from build123d import *

# Parameters (mm, degrees)
SKETCH1_R           = 20.5
BOSS_EXTRUDE1_DEPTH = 25
CHAMFER1_SIZE       = 0.5
SKETCH5_R           = 16.25
CUT_EXTRUDE1_DEPTH  = 20
CHAMFER2_SIZE       = 0.5
SKETCH6_R           = 10.5
CUT_EXTRUDE2_DEPTH  = 31


with BuildPart() as part:
    # Sketch1 → Boss-Extrude1 (new body)
    with BuildSketch(Plane.XY):
        Circle(SKETCH1_R)
    extrude(amount=BOSS_EXTRUDE1_DEPTH)

    # Chamfer1
    chamfer1_edges = [part.edges().sort_by_distance(p)[0] for p in [
        (-20.5, 0, 0),
        (-20.5, 0, 25),
    ]]
    chamfer(chamfer1_edges, length=CHAMFER1_SIZE)

    # Sketch5 → Cut-Extrude1 (cut)
    with BuildSketch(Plane.XY.offset(25)):
        Circle(SKETCH5_R)
    extrude(amount=-CUT_EXTRUDE1_DEPTH, mode=Mode.SUBTRACT)

    # Chamfer2
    chamfer2_edges = [part.edges().sort_by_distance(p)[0] for p in [
        (-16.25, 0, 25),
    ]]
    chamfer(chamfer2_edges, length=CHAMFER2_SIZE)

    # Sketch6 → Cut-Extrude2 (cut)
    with BuildSketch(Plane(origin=(0, 0, 0), x_dir=(-1, 0, 0), z_dir=(0, 0, -1))):
        Circle(SKETCH6_R)
    extrude(amount=-CUT_EXTRUDE2_DEPTH, mode=Mode.SUBTRACT)


solid = part.part
The listing builds one solid part. Answer for the finished solid, in the listing's coordinates (mm). A direction names the side the tool comes from. Coordinates: 2 decimals unless noted, no trailing zeros. Loops run counter-clockwise (first coordinate to the right, second up) from the corner with the lowest first, then second, coordinate; pieces in that order, holes last. Notation, with made-up numbers: (4.5, 17.25) -> (45.5, 17.25) arc R9 cw to (45.5, 31.25) -> close; hole circle Ø11 at (-34.75, -22). An arc over 180 degrees is marked (long way). Answer in a Markdown table with one row per item. Add a question column.
1. The part is cut by section C-C, the plane z = 2.75. Write down the section's boundary in (x, y), then the cut area to 3 significant figures.
2. The part is cut by section D-D, the plane z = 18.25. Write down the section's boundary in (x, y), then the cut area to 3 significant figures.
3. Determine the mould class of faces 1 (the cylindrical face through (-4.444, -20.013, 12.332)), 2 (the flat face through (9, -9, 0)), 3 (the cylindrical face through (15.5, 4.88, 14.89)) for opening direction X: +X half, -X half, draft (parallel to the pull), parting line (faces both ways), or undercut.
4. Consider line 1 (Y direction, x = 0, z = 1); line 2 (Y direction, x = 0, z = 11.5); line 3 (Z direction, x = -14, y = -0.5). Determine where each line is inside the solid, lowest interval first. Write a range as [from, to].
5. For faces 4 (the cylindrical face through (-10, 3.2, 2.5)), 5 (the flat face through (11, 0, 5)), determine the directions among +Z, -Z, +X, -X, +Y, -Y from which every point of the face is accessible in a straight line to the end or side of a thin tool.
6. Flat-ended cylindrical pins translate along their axes: P1, Ø16, axis at x = 2.5, y = -5, coming from the +Z side; P2, Ø5, axis at y = 6, z = 21, coming from the +X side; P3, Ø3, axis at x = 14.5, z = 21, coming from the +Y side; P4, Ø6, axis at x = 16, y = -2, coming from the +Z side. Find the tip coordinate at first contact, or state that the pin passes through.
7. The part is cut by section A-A, the plane y = 0. Write down the section's boundary in (x, z).
Answer below:
| question | item | result |
|---|---|---|
| 1 | outline | circle Ø41 at (0, 0); hole circle Ø21 at (0, 0) |
| 1 | area | 974 mm2 |
| 2 | outline | circle Ø41 at (0, 0); hole circle Ø32.5 at (0, 0) |
| 2 | area | 491 mm2 |
| 3 | face 1 | parting line |
| 3 | face 2 | draft |
| 3 | face 3 | undercut |
| 4 | line 1 | [-20.5, -10.5], [10.5, 20.5] |
| 4 | line 2 | [-20.5, -16.25], [16.25, 20.5] |
| 4 | line 3 | [0, 5] |
| 5 | face 4 | +Z, -Z |
| 5 | face 5 | +Z |
| 6 | P1 | z = 5 |
| 6 | P2 | x = 20.2 |
| 6 | P3 | y = 15.85 |
| 6 | P4 | z = 25 |
| 7 | outline | (-20.5, 0.5) -> (-20, 0) -> (-10.5, 0) -> (-10.5, 5) -> (-16.25, 5) -> (-16.25, 24.5) -> (-16.75, 25) -> (-20, 25) -> (-20.5, 24.5) -> close; (10.5, 0) -> (20, 0) -> (20.5, 0.5) -> (20.5, 24.5) -> (20, 25) -> (16.75, 25) -> (16.25, 24.5) -> (16.25, 5) -> (10.5, 5) -> close |
